Part model, mm, in its own coordinate system. A direction names the side the tool comes from. Round coordinates to 2 decimals unless told otherwise and drop trailing zeros. Loops run counter-clockwise (first coordinate to the right, second up) from the corner with the lowest first, then second, coordinate; pieces in that order, holes last.
(1) Flat gauge pins, fed straight in: pin 1 (8 mm diameter, centred on x = -22.5, y = 435, fed in from -Z); pin 2 (1.5 mm diameter, centred on x = -4, y = -255, fed in from -Z). Where does each tip first touch, or does it go through?
(2) Mould opens along Y. For faces 3 (the face through (0, 6, 2)), 4 (the face through (19, 6, 0)), 5 (the face through (0, 450, 7)) say: +Y half, -Y half, draft (parallel to the pull), parting line (faces both ways), or undercut.
(3) Probe probe 1 along X at (y, z) = (-175, 10); probe 2 along X at (y, z) = (-270, 5); probe 3 along X at (y, z) = (-308.5, 1.5). List the from-to ranges inside material, lowest first.
(4) Cut at A-A on y = 258. List the corners of the cut face in (x, z), then the cut area to 3 significant figures.
(5) Tool access for faces 1 (the face through (0, -435, 3)), 2 (the face through (0, 6, 15)): list every direction of +Z, -Z, +X, -X, +Y, -Y with a clear straight run to the whole face (end or side of a thin tool).
from build123d import *

# Parameters (mm, degrees)
SKETCH1_W           = 60
SKETCH1_H           = 900
BOSS_EXTRUDE1_DEPTH = 15
SKETCH5_W           = 60
SKETCH5_H           = 20
CUT_EXTRUDE2_DEPTH  = 3
SKETCH7_W           = 15
SKETCH7_H           = 850
CUT_EXTRUDE3_DEPTH  = 2
M4_TAPPED_HOLE1_D   = 3.3
LPATTERN1_COUNT     = 14
LPATTERN1_PITCH     = 60
M6_TAPPED_HOLE1_D   = 5
M6_TAPPED_HOLE2_D   = 5
LPATTERN2_COUNT     = 3
LPATTERN2_PITCH     = 175
LPATTERN2_COL_COUNT = 3
LPATTERN2_COL_PITCH = 175


with BuildPart() as part:
    # Sketch1 → Boss-Extrude1 (new body)
    with BuildSketch(Plane.XY):
        Rectangle(SKETCH1_W, SKETCH1_H)
    extrude(amount=BOSS_EXTRUDE1_DEPTH)

    # Sketch5 → Cut-Extrude2 (cut)
    with BuildSketch(Plane(origin=(0, 0, 0), x_dir=(-1, 0, 0), z_dir=(0, 0, -1))):
        with Locations((0, 435)):
            Rectangle(SKETCH5_W, SKETCH5_H)
        with Locations((0, -435)):
            Rectangle(SKETCH5_W, SKETCH5_H)
    extrude(amount=-CUT_EXTRUDE2_DEPTH, mode=Mode.SUBTRACT)

    # Sketch7 → Cut-Extrude3 (cut)
    with BuildSketch(Plane(origin=(0, 0, 0), x_dir=(-1, 0, 0), z_dir=(0, 0, -1))):
        Rectangle(SKETCH7_W, SKETCH7_H)
    extrude(amount=-CUT_EXTRUDE3_DEPTH, mode=Mode.SUBTRACT)

    # M4 Tapped Hole1 (through all)
    with Locations(Plane(origin=(0, 0, 2), x_dir=(-1, 0, 0), z_dir=(0, 0, -1))):
        with Locations((0, 390)):
            m4_tapped_hole1 = Hole(M4_TAPPED_HOLE1_D / 2)

    # LPattern1: M4 Tapped Hole1 ×14
    with Locations(*[(0, -i * LPATTERN1_PITCH, 0) for i in range(1, LPATTERN1_COUNT)]):
        add(m4_tapped_hole1, mode=Mode.SUBTRACT)

    # M6 Tapped Hole1 (through all)
    with Locations(Plane(origin=(0, 0, 3), x_dir=(-1, 0, 0), z_dir=(0, 0, -1))):
        with Locations((-22.5, 435), (22.5, 435), (-22.5, -435), (22.5, -435)):
            Hole(M6_TAPPED_HOLE1_D / 2)

    # M6 Tapped Hole2 (through all)
    with Locations(Plane.XY.offset(15)):
        with Locations((-22.5, 0), (22.5, 0)):
            m6_tapped_hole2 = Hole(M6_TAPPED_HOLE2_D / 2)

    # LPattern2: M6 Tapped Hole2 ×3
    with Locations(*[(0, -i * LPATTERN2_PITCH, 0) for i in range(1, LPATTERN2_COUNT)]):
        add(m6_tapped_hole2, mode=Mode.SUBTRACT)

    # LPattern2 col: M6 Tapped Hole2 ×3
    with Locations(*[(0, i * LPATTERN2_COL_PITCH, 0) for i in range(1, LPATTERN2_COL_COUNT)]):
        add(m6_tapped_hole2, mode=Mode.SUBTRACT)


solid = part.part
Final values:
1. pin 1: stops at z = 3
1. pin 2: stops at z = 2
2. face 3: undercut
2. face 4: draft
2. face 5: +Y half
3. probe 1: x = -30 to -25, -20 to 20, 25 to 30
3. probe 2: x = -30 to -1.65, 1.65 to 30
3. probe 3: x = -30 to -7.5, 7.5 to 30
4. outline: (-30, 0) - (-7.5, 0) - (-7.5, 2) - (7.5, 2) - (7.5, 0) - (30, 0) - (30, 15) - (-30, 15) - close
4. area: 870 mm2
5. face 1: -Z, +X, -X
5. face 2: +Z, +X, -X, +Y, -Y
